```python
from build123d import *

# Parameters (mm, degrees)
DOVETAIL_BASE_SLIDE_DEPTH      = 290
SLOT_COUNTERBORE_10_DEEP_DEPTH = 10
ADJUSTING_SLOT_30_WIDE_DEPTH   = 50
RELIEF_CUT_SKETCH_W            = 120
RELIEF_CUT_SKETCH_H            = 20
RECTANGULAR_RELIEF_CUT_DEPTH   = 50
RAISED_PAD_SKETCH_W            = 120
RAISED_PAD_SKETCH_H            = 120
RAISED_PAD_25_DEPTH            = 25
UPRIGHT_HEAD_DEPTH             = 120
HEAD_THROUGH_SLOT_DEPTH        = 120
HEAD_HOLES_SKETCH_R            = 15
HEAD_HOLES_2X_30_DEPTH         = 120


with BuildPart() as part:
    # Dovetail Base Profile Sketch → Dovetail Base Slide (new body)
    with BuildSketch(Plane.XY):
        Polygon((106.010770255, 40), (106.010770255, 30), (92.021540511, 0), (0, 0), (-13.989229745, 30), (-13.989229745, 40), align=None)
    extrude(amount=-DOVETAIL_BASE_SLIDE_DEPTH)

    # Slot Counterbore Sketch → Slot Counterbore 10 Deep (cut)
    with BuildSketch(Plane(origin=(0, 40, 0), x_dir=(1, 0, 0), z_dir=(0, 1, 0))):
        with BuildLine():
            Line((11.010770255, 120), (11.010770255, 65))
            ThreePointArc((11.010770255, 65), (46.010770255, 30), (81.010770255, 65))
            Line((81.010770255, 65), (81.010770255, 120))
            ThreePointArc((81.010770255, 120), (46.010770255, 155), (11.010770255, 120))
        make_face()
    extrude(amount=-SLOT_COUNTERBORE_10_DEEP_DEPTH, mode=Mode.SUBTRACT)

    # Adjusting Slot Sketch → Adjusting Slot 30 Wide (cut)
    with BuildSketch(Plane(origin=(0, 30, 0), x_dir=(1, 0, 0), z_dir=(0, 1, 0))):
        with BuildLine():
            Line((31.010770255, 120), (31.010770255, 65))
            ThreePointArc((31.010770255, 65), (46.010770255, 50), (61.010770255, 65))
            Line((61.010770255, 65), (61.010770255, 120))
            ThreePointArc((61.010770255, 120), (46.010770255, 135), (31.010770255, 120))
        make_face()
    extrude(amount=-ADJUSTING_SLOT_30_WIDE_DEPTH, mode=Mode.SUBTRACT)

    # Relief Cut Sketch → Rectangular Relief Cut (cut)
    with BuildSketch(Plane(origin=(0, 40, 0), x_dir=(1, 0, 0), z_dir=(0, 1, 0))):
        with Locations((46.010770255, 280)):
            Rectangle(RELIEF_CUT_SKETCH_W, RELIEF_CUT_SKETCH_H)
    extrude(amount=-RECTANGULAR_RELIEF_CUT_DEPTH, mode=Mode.SUBTRACT)

    # Raised Pad Sketch → Raised Pad 25 (add)
    with BuildSketch(Plane(origin=(0, 40, 0), x_dir=(1, 0, 0), z_dir=(0, 1, 0))):
        with Locations((46.010770255, 230)):
            Rectangle(RAISED_PAD_SKETCH_W, RAISED_PAD_SKETCH_H)
    extrude(amount=RAISED_PAD_25_DEPTH)

    # Upright Head Profile Sketch → Upright Head (add)
    with BuildSketch(Plane.XY.offset(-170)):
        Polygon((46.010770255, 140), (6.010770255, 140), (-13.989229745, 65), (106.010770255, 65), (86.010770255, 140), align=None)
    extrude(amount=-UPRIGHT_HEAD_DEPTH)

    # Head Slot Sketch → Head Through Slot (cut)
    with BuildSketch(Plane.XY.offset(-170)):
        with BuildLine():
            Line((23.510770255, 125), (68.510770255, 125))
            ThreePointArc((68.510770255, 125), (83.510770255, 110), (68.510770255, 95))
            Line((68.510770255, 95), (23.510770255, 95))
            ThreePointArc((23.510770255, 95), (8.510770255, 110), (23.510770255, 125))
        make_face()
    extrude(amount=-HEAD_THROUGH_SLOT_DEPTH, mode=Mode.SUBTRACT)

    # Head Holes Sketch → Head Holes 2xØ30 (cut)
    with BuildSketch(Plane.XY.offset(-170)):
        with Locations((18.299617998, 65)):
            Circle(HEAD_HOLES_SKETCH_R)
        with Locations((70.299617998, 65)):
            Circle(HEAD_HOLES_SKETCH_R)
    extrude(amount=-HEAD_HOLES_2X_30_DEPTH, mode=Mode.SUBTRACT)


solid = part.part
```
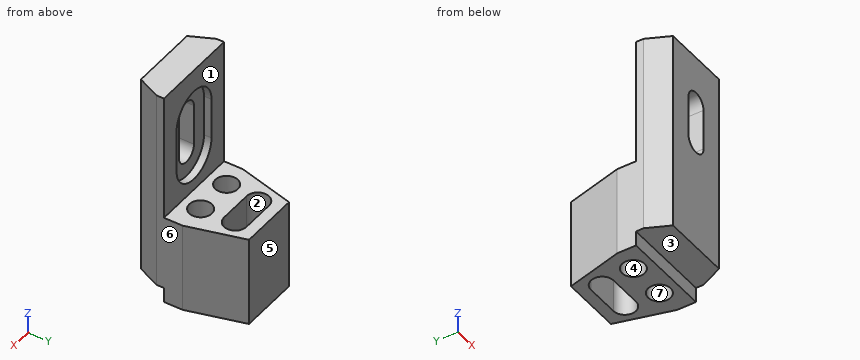
Model file for the job. Use its own axes, mm. Face numbers are marked on the shaded views. A direction names the side the tool comes from. Round coordinates to 2 decimals unless told otherwise and drop trailing zeros. Write each loop counter-clockwise with the first axis right and the second up, starting at its lowest first coordinate (ties: lowest second). Pieces come first, ordered by that corner, then holes. Notation, with made-up numbers: (-13.75, 67) -> (23.25, 67) arc R24 ccw to (23.25, 87) -> close; hole circle Ø5 at (10.25, 12.25). An arc over 180 degrees is marked (long way). Answer as CSV lines item,"result".
1. Pin check, flat tips, straight feed: pin 1 Ø9 at (y, z) = (12, -97) entering from +X; pin 2 Ø16 at (x, z) = (67, -283) entering from -Y; pin 3 Ø3 at (x, z) = (48.5, -134) entering from +Y; pin 4 Ø24 at (x, y) = (70.3, 65) entering from +Z. Stop position of each tip, or through.
Resolved:
pin 1,"x = 99.72"
pin 2,"y = 40"
pin 3,"y = 30"
pin 4,"through"
2. Drill centre lines: line 1 (Y direction, x = 69.5, z = -277); line 2 (Y direction, x = 23.5, z = -258.5); line 3 (X direction, y = 67.5, z = -261.5). Where is each one in solid material? Low to high.
Resolved:
line 1,"40 to 50.02, 79.98 to 95.03, 124.97 to 140"
line 2,"0 to 50.93, 79.07 to 95, 125 to 140"
line 3,"-13.32 to 3.51, 33.09 to 55.51, 85.09 to 105.34"
3. Mould opens along X. For the marked faces 4, 5, 6 and 7 say: +X half, -X half, draft (parallel to the pull), parting line (faces both ways), or undercut.
Resolved:
face 4,"undercut"
face 5,"draft"
face 6,"+X half"
face 7,"undercut"
4. Slice it at A-A, the plane z = -112. List the corners of the cut face in (x, y).
Resolved:
outline,"(-13.99, 30) -> (0, 0) -> (31.01, 0) -> (31.01, 30) -> (11.01, 30) -> (11.01, 40) -> (-13.99, 40) -> close; (61.01, 0) -> (92.02, 0) -> (106.01, 30) -> (106.01, 40) -> (81.01, 40) -> (81.01, 30) -> (61.01, 30) -> close"
5. Slice it at D-D, the plane z = -199. List the corners of the cut face in (x, y).
Resolved:
outline,"(-13.99, 30) -> (0, 0) -> (92.02, 0) -> (106.01, 30) -> (106.01, 65) -> (86.01, 140) -> (6.01, 140) -> (-13.99, 65) -> close; hole circle Ø30 at (18.3, 65); hole (23.51, 95) -> (68.51, 95) arc R15 ccw to (68.51, 125) -> (23.51, 125) arc R15 ccw to start; hole circle Ø30 at (70.3, 65)"
6. Tool access for the marked faces 1, 2 and 3: list every direction of +Z, -Z, +X, -X, +Y, -Y with a clear straight run to the whole face (end or side of a thin tool).
Resolved:
face 1,"+Z, +X, -X, +Y"
face 2,"+Z, -Z"
face 3,"-Z, +X, -X, -Y"
7. Slice it at C-C, the plane y = 116. List the corners of the cut face in (x, z).
Resolved:
outline,"(-0.39, -290) -> (9.76, -290) -> (9.76, -170) -> (-0.39, -170) -> close; (82.26, -290) -> (92.41, -290) -> (92.41, -170) -> (82.26, -170) -> close"
8. Slice it at B-B, the plane x = 14. List the corners of the cut face in (y, z).
Resolved:
outline,"(0, -270) -> (40, -270) -> (40, -290) -> (50.63, -290) -> (50.63, -170) -> (40, -170) -> (40, -134.15) -> (30, -134.15) -> (30, -50.85) -> (40, -50.85) -> (40, 0) -> (0, 0) -> close; (79.37, -290) -> (98.4, -290) -> (98.4, -170) -> (79.37, -170) -> close; (121.6, -290) -> (140, -290) -> (140, -170) -> (121.6, -170) -> close"
